Part print with two shaded views. Sizes in mm from the minimum x, y, z corner. Round coordinates to 2 decimals unless told otherwise and drop trailing zeros. Write each loop counter-clockwise with the first axis right and the second up, starting at its lowest first coordinate (ties: lowest second). Pieces come first, ordered by that corner, then holes. Notation, with made-up numbers: (67, 64.5) - (103, 64.5) arc R24 cw to (103, 83.5) - close; hole circle Ø5 at (-18.75, 11.25). An arc over 180 degrees is marked (long way). Answer as a JSON object with one key per item and string values. Group by question number.
Item 1: Slice it at A-A, the plane z = 55. List the corners of the cut face in (x, y).
Item 2: Slice it at C-C, the plane y = 2.25. List the corners of the cut face in (x, z), then the cut area to 3 significant figures.
Item 3: Flat gauge pins, fed straight in: pin 1 (1.5 mm diameter, centred on x = 27, y = 7, fed in from +Z); pin 2 (2 mm diameter, centred on x = 21, y = 2, fed in from -Z); pin 3 (3 mm diameter, centred on y = 3, z = 85.5, fed in from +X). Where does each tip first touch, or does it go through?
Item 4: Probe line 1 (Z direction, x = 55, y = 4.1); line 2 (X direction, y = 5, z = 64.5). List the from-to ranges inside material, lowest first. Write a range as from..to.
Item 5: Slice it at B-B, the plane x = 55. List the corners of the cut face in (y, z), then the cut area to 3 significant figures.
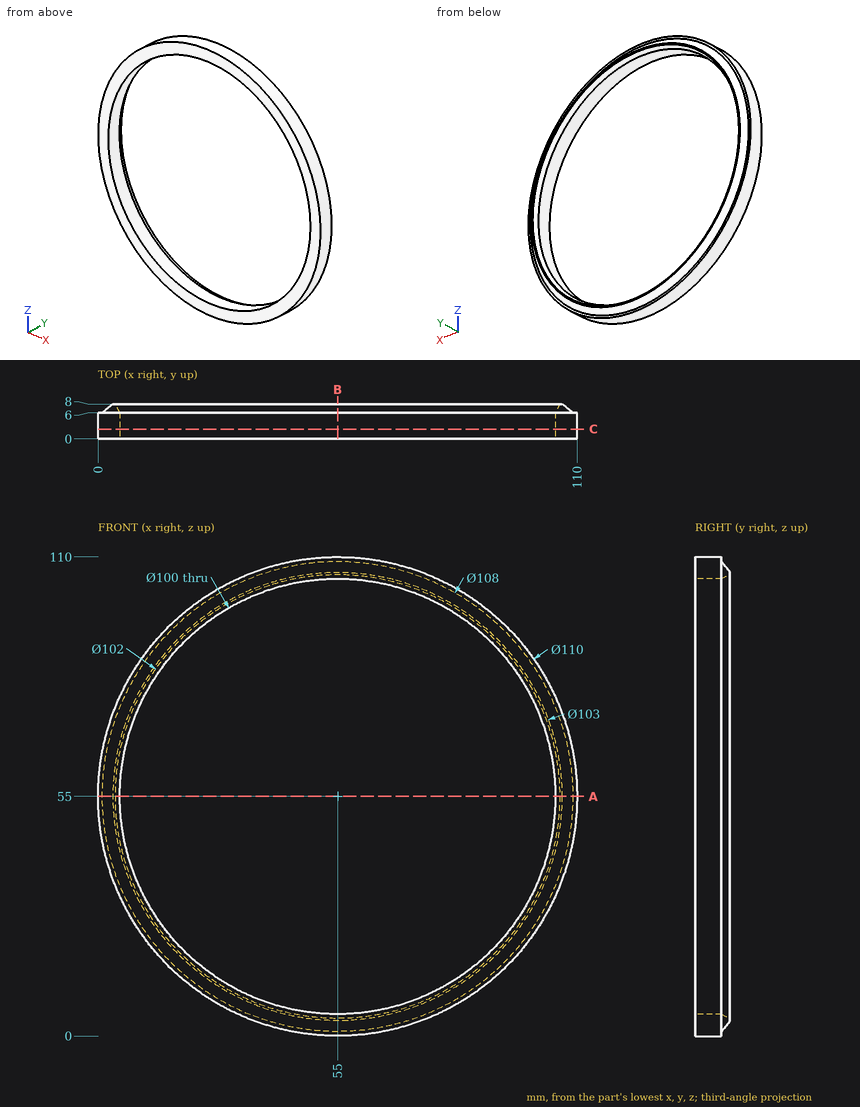
Geometry says:
{
 "1": {"outline": "(0, 0) - (5, 0) - (5, 6) - (4, 8) - (3.5, 8) - (1, 6) - (0, 6) - close; (105, 0) - (110, 0) - (110, 6) - (109, 6) - (106.5, 8) - (106, 8) - (105, 6) - close"},
 "2": {"outline": "circle Ø110 at (55, 55); hole circle Ø100 at (55, 55)", "area": "1,650 mm^2"},
 "3": {"pin 1": "stops at z = 100.9", "pin 2": "stops at z = 11", "pin 3": "stops at x = 101.73"},
 "4": {"line 1": "z = 0..5, 105..110", "line 2": "x = 0.83..5.91, 104.09..109.17"},
 "5": {"outline": "(0, 0) - (6, 0) - (6, 1) - (8, 3.5) - (8, 4) - (6, 5) - (0, 5) - close; (0, 105) - (6, 105) - (8, 106) - (8, 106.5) - (6, 109) - (6, 110) - (0, 110) - close", "area": "69.0 mm^2"}
}
